from build123d import *

# Parameters (mm, degrees)
SKETCH_1_W                  = 43
SKETCH_1_H                  = 32
EXTRUDE_1_DEPTH             = 3
HOLE_WIZARD_M5_1_AT_2_COUNT = 2
HOLE_WIZARD_M5_1_AT_2_PITCH = 30
SKETCH_4_R                  = 3.25
CUT_EXTRUDE_1_DEPTH         = 3
FILLET_1_R                  = 2
SKETCH_5_R                  = 2.75
EXTRUDE_2_DEPTH             = 10


with BuildPart() as part:
    # 草图1 → 凸台-拉伸1 (new body)
    with BuildSketch(Plane.XY):
        with Locations((21.5, -16)):
            Rectangle(SKETCH_1_W, SKETCH_1_H)
    extrude(amount=EXTRUDE_1_DEPTH)

    # 草图2 → M5 六角凹锥坑螺钉的锥形沉头孔1 (revolve, cut)
    with BuildSketch(Plane(origin=(6.5, -7, 3), x_dir=(0, -1, 0), z_dir=(1, 0, 0))):
        Polygon((0, 0), (0, 3), (2.75, 3), (2.75, 2.85), (5.6, 0), align=None)
    hole_wizard_m5_1 = revolve(axis=Axis((6.5, -7, 9.35), (0, 0, -1)), mode=Mode.SUBTRACT)

    # M5 六角凹锥坑螺钉的锥形沉头孔1 at 2: M5 六角凹锥坑螺钉的锥形沉头孔1 ×2
    with Locations(*[(i * HOLE_WIZARD_M5_1_AT_2_PITCH, 0, 0) for i in range(1, HOLE_WIZARD_M5_1_AT_2_COUNT)]):
        add(hole_wizard_m5_1, mode=Mode.SUBTRACT)

    # 草图4 → 切除-拉伸1 (cut)
    with BuildSketch(Plane.XY.offset(3)):
        with Locations((21.5, -27)):
            Circle(SKETCH_4_R)
    extrude(amount=-CUT_EXTRUDE_1_DEPTH, mode=Mode.SUBTRACT)

    # 圆角1
    fillet_1_edges = [part.edges().sort_by_distance(p)[0] for p in [
        (0, 0, 1.5),
        (43, 0, 1.5),
        (43, -32, 1.5),
        (0, -32, 1.5),
    ]]
    fillet(fillet_1_edges, radius=FILLET_1_R)

    # 草图5 → 凸台-拉伸2 (add)
    with BuildSketch(Plane(origin=(0, 0, 0), x_dir=(-1, 0, 0), z_dir=(0, 0, -1))):
        with BuildLine():
            Line((-43, -2), (-43, -12))
            Line((-43, -12), (0, -12))
            Line((0, -12), (0, -2))
            ThreePointArc((0, -2), (-0.585786438, -0.585786438), (-2, 0))
            Line((-2, 0), (-41, 0))
            ThreePointArc((-41, 0), (-42.414213562, -0.585786438), (-43, -2))
        make_face()
        with Locations(Location((-36.5, -7, 0), (0, 0, 180))):
            Circle(SKETCH_5_R, mode=Mode.SUBTRACT)
        with Locations(Location((-6.5, -7, 0), (0, 0, 180))):
            Circle(SKETCH_5_R, mode=Mode.SUBTRACT)
    extrude(amount=EXTRUDE_2_DEPTH)


solid = part.part
Model file for the job. Use its own axes, mm. A direction names the side the tool comes from. Give positions to 0.01 mm unless a question says otherwise; leave off trailing zeros. Order: outer loops, then holes, each group sorted by start corner. A loop starts at its lowest first (then second) coordinate and runs counter-clockwise, first axis right, second up. Notation, with made-up numbers: M 14,11 L 55,11 A30 cw 55,43 Z; hole C -36,13 d4. An arc over 180 degrees is marked long. Put each result on its own line as item: value. Start each with the question number.
(1) Pull direction X, two halves, no side cores. Call faces 1 (the face through (34.031, -8.574, 0.328)), 2 (the face through (0.57, -0.6, -3.41)), 3 (the face through (21, -32, 1)): released by +X, released by -X, zero draft, split by the parting line, or undercut.
(2) Band-saw the part on C-C on x = 21.5. Give the cut face in (y, z).
(3) Tool access for faces 4 (the face through (22, -12, -5)), 5 (the face through (9.052, -8.023, -4.854)): list every direction of +Z, -Z, +X, -X, +Y, -Y with a clear straight run to the whole face (end or side of a thin tool).
(4) Drill centre lines: L1, parallel to X at y = -7, z = -3; L2, parallel to Y at x = 21.5, z = 1.2; L3, parallel to Y at x = 36.5, z = -3.5. Where is each one in solid material? Low to high. Write a range as [from, to].
(5) Pin check, flat tips, straight feed: pin 1 Ø5 at (x, z) = (9, -5) entering from -Y; pin 2 Ø6.5 at (x, y) = (6.5, -7) entering from +Z; pin 3 Ø4 at (x, y) = (21.5, -27) entering from -Z. Stop position of each tip, or through.
(6) Band-saw the part on B-B on y = -27. Give the cut face in (x, z), then the cut area to 4 significant figures.
(7) Band-saw the part on A-A on z = 0.75. Give the cut face in (x, y), then the cut area to 3 significant figures.
(8) Band-saw the part on D-D on x = 29. Give the cut face in (y, z), then the cut area to 3 significant figures.
Results below:
1. face 1: undercut
1. face 2: released by -X
1. face 3: zero draft
2. outline: M -32,0 L -30.25,0 L -30.25,3 L -32,3 Z; M -23.75,0 L -12,0 L -12,-10 L 0,-10 L 0,3 L -23.75,3 Z
3. face 4: -Z, +X, -X, -Y
3. face 5: +Z, -Z
4. L1: x = [0, 3.75], [9.25, 33.75], [39.25, 43]
4. L2: y = [-32, -30.25], [-23.75, 0]
4. L3: y = [-12, -9.75], [-4.25, 0]
5. pin 1: stops at y = -12
5. pin 2: stops at z = 0.65
5. pin 3: passes through
6. outline: M 0,0 L 18.25,0 L 18.25,3 L 0,3 Z; M 24.75,0 L 43,0 L 43,3 L 24.75,3 Z
6. area: 109.5 mm2
7. outline: M 0,-30 A2 ccw 2,-32 L 41,-32 A2 ccw 43,-30 L 43,-2 A2 ccw 41,0 L 2,0 A2 ccw 0,-2 Z; hole C 6.5,-7 d6.7; hole C 21.5,-27 d6.5; hole C 36.5,-7 d6.7
7. area: 1,270 mm2
8. outline: M -32,0 L -12,0 L -12,-10 L 0,-10 L 0,3 L -32,3 Z
8. area: 216 mm2
